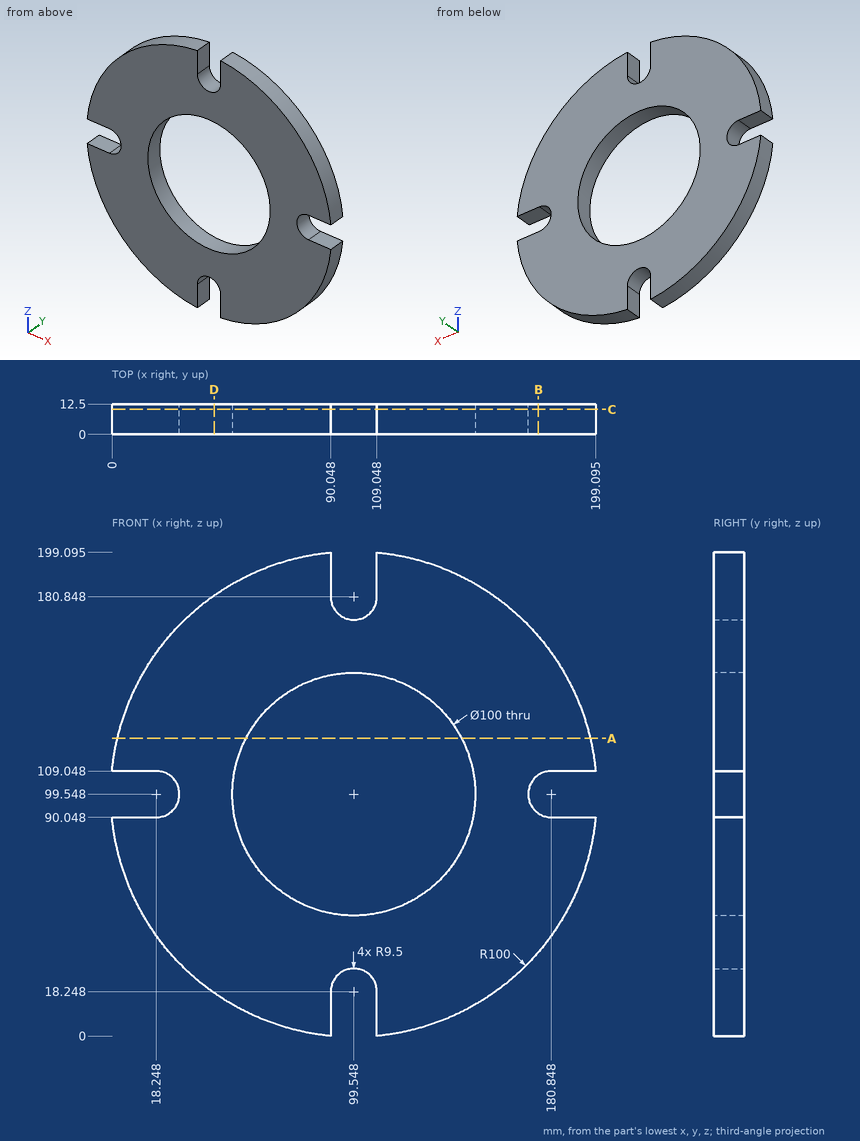
Geometry: see drawing. Coordinates: mm, zero at the bounding-box minimum. Round coordinates to 2 decimals unless told otherwise and drop trailing zeros. Loops run counter-clockwise (first coordinate to the right, second up) from the corner with the lowest first, then second, coordinate; pieces in that order, holes last. Notation, with made-up numbers: M 75,47.25 L 133,47.25 A13 ccw 133,53.25 Z; hole C 58.5,50 d11. An arc over 180 degrees is marked long. Use a Markdown table: item, result. Add a question column.
1. Section query B-B on x = 175.5. Return the cut outline in (y, z) (1 decimal), then the cut area to 3 significant figures.
2. Section query A-A on z = 122.5. Return the cut outline in (x, y).
3. Section query D-D on x = 42. Return the cut outline in (y, z).
4. Contact query for flat-ended pins moving along their axis: P1, Ø1.5, axis at x = 75, y = 8, coming from the -Z side; P2, Ø6, axis at x = 192, y = 3.5, coming from the +Z side; P3, Ø4, axis at y = 9.5, z = 192, coming from the +X side. Output: stop coordinate, or through.
5. Line query: line 1 (X direction, y = 10.75, z = 91) (1 decimal); line 2 (Z direction, x = 21.5, y = 8.75) (1 decimal); line 3 (X direction, y = 9, z = 64.5) (1 decimal). Output: solid intervals per line, ascending.
6. Section query C-C on y = 10.25. Return the cut outline in (x, z) (1 decimal).
Reported:
| question | item | result |
|---|---|---|
| 1 | outline | M 0,34.5 L 12.5,34.5 L 12.5,91.7 L 0,91.7 Z; M 0,107.4 L 12.5,107.4 L 12.5,164.6 L 0,164.6 Z |
| 1 | area | 1,430 mm² |
| 2 | outline | M 2.22,0 L 55.13,0 L 55.13,12.5 L 2.22,12.5 Z; M 143.97,0 L 196.88,0 L 196.88,12.5 L 143.97,12.5 Z |
| 3 | outline | M 0,17.77 L 12.5,17.77 L 12.5,181.33 L 0,181.33 Z |
| 4 | P1 | stops at z = 2.42 |
| 4 | P2 | stops at z = 144.25 |
| 4 | P3 | stops at x = 142.19 |
| 5 | line 1 | x = 22.4 to 50.3, 148.8 to 176.7 |
| 5 | line 2 | z = 37 to 90.6, 108.5 to 162.1 |
| 5 | line 3 | x = 5.9 to 63.9, 135.2 to 193.2 |
| 6 | outline | M 0,90 A100 ccw 90,0 L 90,18.2 A9.5 cw 109,18.2 L 109,0 A100 ccw 199.1,90 L 180.8,90 A9.5 cw 180.8,109 L 199.1,109 A100 ccw 109,199.1 L 109,180.8 A9.5 cw 90,180.8 L 90,199.1 A100 ccw 0,109 L 18.2,109 A9.5 cw 18.2,90 Z; hole C 99.5,99.5 d100 |
